The figure shows three views and two pictorial views of one solid part (mm, origin at its lowest corner). Answer the questions. Coordinates: 2 decimals unless noted, no trailing zeros. Order: outer loops, then holes, each group sorted by start corner. A loop starts at its lowest first (then second) coordinate and runs counter-clockwise, first axis right, second up. Notation, with made-up numbers: (14.5, 5.5) - (34.5, 5.5) arc R19 ccw to (34.5, 41.5) - close; hole circle Ø6 at (22, 41.25). An arc over 180 degrees is marked (long way). Use one line per item in the form item = value. Start each with the question number.
Item 1: Section B-B, the plane x = 5.75 is taken. Write down the section's boundary in (y, z), and give its area (3 significant figures).
Item 2: Each of these flat-tipped pins is pushed along its axis until it touches: pin 1 Ø3.5 at (x, y) = (7, 50) entering from +Z; pin 2 Ø1 at (x, y) = (9.5, 66) entering from -Z. Where does it stop, or does it pass through?
Item 3: Section C-C, the plane y = 148 is taken. Write down the section's boundary in (x, z).
Item 4: Consider line 1 along Y through (x, z) = (1.5, 132); line 2 along Y through (x, z) = (8.25, 36.5); line 3 along Z through (x, y) = (1, 153). Determine where each line is inside the solid, lowest interval first. Write a range as [from, to].
Item 5: Section A-A, the plane z = 141.5 is taken. Write down the section's boundary in (x, y), and give its area (3 significant figures).
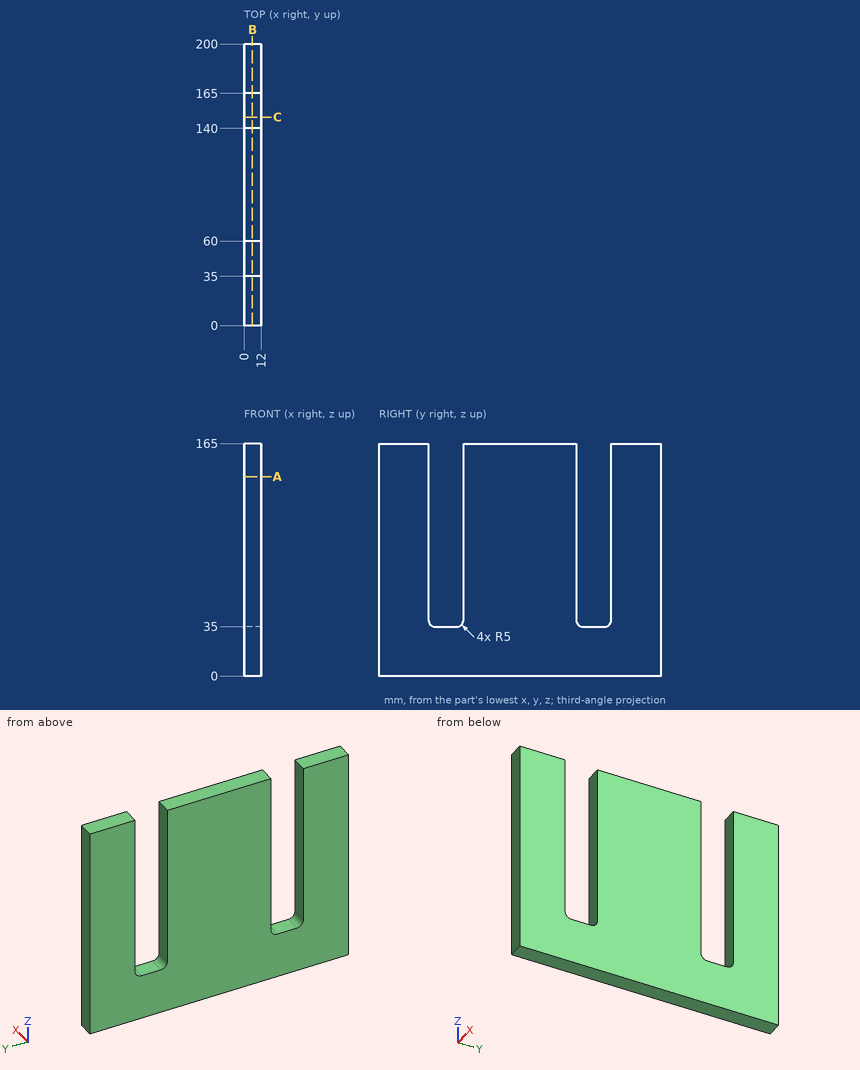
Response:
q1.outline = (0, 0) - (200, 0) - (200, 165) - (165, 165) - (165, 40) arc R5 cw to (160, 35) - (145, 35) arc R5 cw to (140, 40) - (140, 165) - (60, 165) - (60, 40) arc R5 cw to (55, 35) - (40, 35) arc R5 cw to (35, 40) - (35, 165) - (0, 165) - close
q1.area = 26,500 mm2
q2.pin_1 = 35
q2.pin_2 = 0
q3.outline = (0, 0) - (12, 0) - (12, 35) - (0, 35) - close
q4.line_1 = [0, 35], [60, 140], [165, 200]
q4.line_2 = [0, 36.43], [58.57, 141.43], [163.57, 200]
q4.line_3 = [0, 35]
q5.outline = (0, 0) - (12, 0) - (12, 35) - (0, 35) - close; (0, 60) - (12, 60) - (12, 140) - (0, 140) - close; (0, 165) - (12, 165) - (12, 200) - (0, 200) - close
q5.area = 1,800 mm2
